```python
from build123d import *

# Parameters (mm, degrees)
SKETCH_1_W         = 18
SKETCH_1_H         = 6
EXTRUDE_1_DEPTH    = 10
HOLE_WIZARD_M4_3_D = 3.3
FILLET_1_R         = 2


with BuildPart() as part:
    # 草图1 → 凸台-拉伸1 (new body)
    with BuildSketch(Plane.XY):
        Rectangle(SKETCH_1_W, SKETCH_1_H)
    extrude(amount=EXTRUDE_1_DEPTH)

    # M4 螺纹孔3 (through all)
    with Locations(Plane(origin=(0, 3, 0), x_dir=(1, 0, 0), z_dir=(0, 1, 0))):
        with Locations((6, -5), (-6, -5)):
            Hole(HOLE_WIZARD_M4_3_D / 2)

    # 圆角1
    fillet_1_edges = [part.edges().sort_by_distance(p)[0] for p in [
        (-9, 0, 10),
        (9, 0, 10),
        (-9, 0, 0),
        (9, 0, 0),
    ]]
    fillet(fillet_1_edges, radius=FILLET_1_R)


solid = part.part
```
Verification items for the finished model (mm, model axes). Round coordinates to 2 decimals unless told otherwise and drop trailing zeros. Order: outer loops, then holes, each group sorted by start corner. A loop starts at its lowest first (then second) coordinate and runs counter-clockwise, first axis right, second up. Notation, with made-up numbers: (38, -36) - (75, -36) arc R17 ccw to (75, -23) - close; hole circle Ø2 at (16, -27). An arc over 180 degrees is marked (long way). Use CSV: the item, a comma, the result in double quotes. Start each with the question number.
1) Section check D-D, the plane z = 4. Record the cut outline in (x, y).
2) Mould release check, pull along X, two halves, no side actions. Record for faces 1 (the cylindrical face through (-4.35, -0.04, 4.93)), 2 (the cylindrical face through (7.65, -0.04, 4.93)), 3 (the cylindrical face through (8.4, 0.04, 9.43)), 4 (the flat face through (0, 3, 5)): +X half, -X half, draft (parallel to the pull), parting line (faces both ways), or undercut.
3) Section check C-C, the plane y = 0.6. Record the cut outline in (x, z), plus the area to 3 significant figures.
4) Thickness scan on L1, parallel to X at y = 1.65, z = 5; L2, parallel to Z at x = 6, y = -0.9; L3, parallel to Z at x = 7, y = 1.1. Record the ranges inside material, lowest first.
5) Go/stop test with flat-tipped pins: P1, Ø1.5, axis at y = 1, z = 9, coming from the -X side; P2, Ø2.5, axis at x = 6, z = 5, coming from the +Y side. Record where each tip stops, or that it passes through.
6) Section check A-A, the plane z = 5. Record the cut outline in (x, y).
7) Section check B-B, the plane x = 6. Record the cut outline in (y, z), plus the area to 3 significant figures.
Answers:
1,outline,"(-9, -3) - (-7.31, -3) - (-7.31, 3) - (-9, 3) - close; (-4.69, -3) - (4.69, -3) - (4.69, 3) - (-4.69, 3) - close; (7.31, -3) - (9, -3) - (9, 3) - (7.31, 3) - close"
2,face 1,"undercut"
2,face 2,"undercut"
2,face 3,"+X half"
2,face 4,"draft"
3,outline,"(-9, 2) arc R2 ccw to (-7, 0) - (7, 0) arc R2 ccw to (9, 2) - (9, 8) arc R2 ccw to (7, 10) - (-7, 10) arc R2 ccw to (-9, 8) - close; hole circle Ø3.3 at (-6, 5); hole circle Ø3.3 at (6, 5)"
3,area,"159 mm²"
4,L1,"x = -9 to -7.65, -4.35 to 4.35, 7.65 to 9"
4,L2,"z = 0 to 3.35, 6.65 to 10"
4,L3,"z = 0 to 3.69, 6.31 to 10"
5,P1,"stops at x = -8.98"
5,P2,"passes through"
6,outline,"(-9, -3) - (-7.65, -3) - (-7.65, 3) - (-9, 3) - close; (-4.35, -3) - (4.35, -3) - (4.35, 3) - (-4.35, 3) - close; (7.65, -3) - (9, -3) - (9, 3) - (7.65, 3) - close"
7,outline,"(-3, 0) - (3, 0) - (3, 3.35) - (-3, 3.35) - close; (-3, 6.65) - (3, 6.65) - (3, 10) - (-3, 10) - close"
7,area,"40.2 mm²"
